```python
from build123d import *

# Parameters (mm, degrees)
BOSS_EXTRUDE2_DEPTH = 300
FILLET3_R           = 20
FILLET4_R           = 50
FILLET5_R           = 20
SKETCH2_R           = 112.5
SKETCH2_R_2         = 87.5
BOSS_EXTRUDE3_DEPTH = 170
CUT_EXTRUDE1_REACH  = 612.139
SKETCH3_R           = 37.5
CUT_EXTRUDE2_REACH  = 624.454
SKETCH4_R           = 25


with BuildPart() as part:
    # Sketch1 → Boss-Extrude2 (new body)
    with BuildSketch(Plane.XY):
        Polygon((187.5, 0), (-187.5, 0), (-187.5, 238), (-475, 238), (-475, 208), (-217.5, 208), (-217.5, -30), (217.5, -30), (217.5, 208), (475, 208), (475, 238), (187.5, 238), align=None)
    extrude(amount=BOSS_EXTRUDE2_DEPTH)

    # Fillet3
    fillet3_edges = [part.edges().sort_by_distance(p)[0] for p in [
        (-187.5, 0, 150),
        (187.5, 0, 150),
    ]]
    fillet(fillet3_edges, radius=FILLET3_R)

    # Fillet4
    fillet4_edges = [part.edges().sort_by_distance(p)[0] for p in [
        (187.5, 238, 150),
        (217.5, -30, 150),
        (-217.5, -30, 150),
        (-187.5, 238, 150),
    ]]
    fillet(fillet4_edges, radius=FILLET4_R)

    # Fillet5
    fillet5_edges = [part.edges().sort_by_distance(p)[0] for p in [
        (217.5, 208, 150),
        (-217.5, 208, 150),
    ]]
    fillet(fillet5_edges, radius=FILLET5_R)

    # Sketch2 → Boss-Extrude3 (add)
    with BuildSketch(Plane(origin=(0, 0, 0), x_dir=(1, 0, 0), z_dir=(0, 1, 0))):
        with Locations((0, -150)):
            Circle(SKETCH2_R)
        with Locations(Location((0, -150, 0), (0, 0, 180))):
            Circle(SKETCH2_R_2, mode=Mode.SUBTRACT)
    extrude(amount=BOSS_EXTRUDE3_DEPTH)

    # Sketch3 → Cut-Extrude1 (cut, up to next)
    with BuildSketch(Plane(origin=(0, 0, 0), x_dir=(1, 0, 0), z_dir=(0, 1, 0)), mode=Mode.PRIVATE) as cut_extrude1_sk1:
        with Locations(Location((0, -150, 0), (0, 0, 180))):
            Circle(SKETCH3_R)
    cut_extrude1_tool1 = extrude(cut_extrude1_sk1.sketch, amount=-CUT_EXTRUDE1_REACH, mode=Mode.PRIVATE) & part.part
    add(cut_extrude1_tool1.solids().sort_by_distance((0, 0, 150))[0], mode=Mode.SUBTRACT)

    # Sketch4 → Cut-Extrude2 (cut, up to next)
    with BuildSketch(Plane(origin=(0, 238, 0), x_dir=(1, 0, 0), z_dir=(0, 1, 0)), mode=Mode.PRIVATE) as cut_extrude2_sk1:
        with Locations(Location((-356.25, -150, 0), (0, 0, 180))):
            Circle(SKETCH4_R)
    cut_extrude2_tool1 = extrude(cut_extrude2_sk1.sketch, amount=-CUT_EXTRUDE2_REACH, mode=Mode.PRIVATE) & part.part
    # Sketch4 → Cut-Extrude2 (cut, up to next)
    with BuildSketch(Plane(origin=(0, 238, 0), x_dir=(1, 0, 0), z_dir=(0, 1, 0)), mode=Mode.PRIVATE) as cut_extrude2_sk2:
        with Locations(Location((355, -150, 0), (0, 0, 180))):
            Circle(SKETCH4_R)
    cut_extrude2_tool2 = extrude(cut_extrude2_sk2.sketch, amount=-CUT_EXTRUDE2_REACH, mode=Mode.PRIVATE) & part.part
    add(cut_extrude2_tool1.solids().sort_by_distance((-356.25, 238, 150))[0], mode=Mode.SUBTRACT)
    add(cut_extrude2_tool2.solids().sort_by_distance((355, 238, 150))[0], mode=Mode.SUBTRACT)


solid = part.part
```
Read the model definition and answer for the solid it produces. Units are mm, in the model's axes. A direction names the side the tool comes from. Coordinates: 2 decimals unless noted, no trailing zeros. Write each loop counter-clockwise with the first axis right and the second up, starting at its lowest first coordinate (ties: lowest second). Pieces come first, ordered by that corner, then holes. Notation, with made-up numbers: (55, 17) - (63, 17) arc R24 ccw to (63, 42) - close; hole circle Ø4 at (76.5, 59). An arc over 180 degrees is marked (long way). Answer as a JSON object with one key per item and string values. Group by question number.
1. A cutting plane is placed at D-D (z = 150). Give the number of separate pieces and of enclosed holes in the cut face, plus the area to 3 significant figures.
2. A cutting plane is placed at B-B (y = 79). Determine the outline of the cut face in (x, z).
3. Each of these flat-tipped pins is pushed along its axis until it touches: P1, Ø1.5, axis at y = 142.5, z = 208.5, coming from the +X side; P2, Ø1, axis at x = 144, z = 53, coming from the +Y side; P3, Ø2, axis at y = 113.5, z = 106.5, coming from the -X side. Where does it stop, or does it pass through?
4. A cutting plane is placed at A-A (x = 0). Determine the outline of the cut face in (y, z), plus the area to 4 significant figures.
5. A cutting plane is placed at C-C (y = 178.5). Determine the outline of the cut face in (x, z).
6. The mould has two halves that part along X. Classify faces 1 (the flat face through (217.5, 103, 148)), 2 (the flat face through (187.5, 105, 148)), 3 (the cylindrical face through (-223.514, 202.297, 152.1)): +X half, -X half, draft (parallel to the pull), parting line (faces both ways), or undercut.
7. Which of the six approach directions +Z, -Z, +X, -X, +Y, -Y give full straight-line access (tool end or side, diameter ignored) to faces 4 (the flat face through (328, 208, 148)), 5 (the flat face through (-217.5, 105, 148)), 6 (the cylindrical face through (18.97, 83.81, 64.58)), 7 (the flat face through (58, 170, 216))?
8. Consider L1, parallel to Z at x = -356.25, y = 227; L2, parallel to Z at x = 0, y = -17; L3, parallel to X at y = 190, z = 111. Determine where each line is inside the solid, lowest interval first. Write a range as [from, to].
Worked out:
{
 "1": {"separate pieces": "4", "enclosed holes": "0", "area": "44,200 mm²"},
 "2": {"outline": "(-217.5, 0) - (-187.5, 0) - (-187.5, 300) - (-217.5, 300) - close; circle Ø225 at (0, 150); (187.5, 0) - (217.5, 0) - (217.5, 300) - (187.5, 300) - close; hole circle Ø175 at (0, 150)"},
 "3": {"P1": "stops at x = 217.5", "P2": "stops at y = 0", "P3": "stops at x = -217.5"},
 "4": {"outline": "(-30, 0) - (0, 0) - (0, 37.5) - (170, 37.5) - (170, 62.5) - (0, 62.5) - (0, 112.5) - (-30, 112.5) - close; (-30, 187.5) - (0, 187.5) - (0, 237.5) - (170, 237.5) - (170, 262.5) - (0, 262.5) - (0, 300) - (-30, 300) - close", "area": "15,250 mm²"},
 "5": {"outline": "(-217.5, 0) - (-187.5, 0) - (-187.5, 300) - (-217.5, 300) - close; (187.5, 0) - (217.5, 0) - (217.5, 300) - (187.5, 300) - close"},
 "6": {"face 1": "+X half", "face 2": "undercut", "face 3": "-X half"},
 "7": {"face 4": "+Z, -Z, +X, -Y", "face 5": "+Z, -Z, -X, -Y", "face 6": "+Y", "face 7": "+Z, -Z, +Y"},
 "8": {"L1": "z = [0, 125], [175, 300]", "L2": "z = [0, 112.5], [187.5, 300]", "L3": "x = [-217.6, -187.54], [187.54, 217.6]"}
}
